Can you work these out from the model? Positions are in its coordinate system, mm. Coordinates: 2 decimals unless noted, no trailing zeros. Loops run counter-clockwise (first coordinate to the right, second up) from the corner with the lowest first, then second, coordinate; pieces in that order, holes last. Notation, with made-up numbers: M -1,17.25 L 57,17.25 A24 cw 57,28.25 Z; hole C 5.5,-11 d9. An arc over 180 degrees is marked long. Answer as a JSON object with one key per item and string values. Group by question number.
Item 1: Suppose I cut it at B-B (z = 21). Write out the boundary of the cut face in (x, y), then the cut area to 3 significant figures.
Item 2: If I drill on line 1 (X direction, y = 1.35, z = 21); line 2 (Y direction, x = 16.5, z = 22.5), over which ranges is the centre line in solid material (lowest first)?
Item 3: I'm going to push a flat-ended pin straight in: pin 1 Ø4.5 at (x, z) = (15, 21) entering from +Y. Where does the tip first touch, or does it pass through?
Item 4: Suppose I cut it at C-C (y = 0.85). Write out the boundary of the cut face in (x, z).
Item 5: We'd pull the mould along Z, two halves only. Please class faces 1 (the flat face through (0, 1, 25.75)), 2 (the cylindrical face through (16.18, 0.89, -22.29)), 3 (the flat face through (-24.75, 1, 0)): +Z half, -Z half, draft (parallel to the pull), parting line (faces both ways), or undercut.
Item 6: Suppose I cut it at A-A (x = 15). Write out the boundary of the cut face in (y, z).
```python
from build123d import *

# Parameters (mm, degrees)
SKETCH1_W           = 49.5
SKETCH1_H           = 51.5
SKETCH1_R           = 1.75
BOSS_EXTRUDE1_DEPTH = 3
CHAMFER1_SIZE       = 1.2
FILLET1_R           = 3


with BuildPart() as part:
    # Sketch1 → Boss-Extrude1 (new body)
    with BuildSketch(Plane(origin=(0, 0, 0), x_dir=(1, 0, 0), z_dir=(0, 1, 0))):
        Rectangle(SKETCH1_W, SKETCH1_H)
        with Locations(Location((-15, 21, 0), (0, 0, 270))):
            Circle(SKETCH1_R, mode=Mode.SUBTRACT)
        with Locations(Location((15, 21, 0), (0, 0, 270))):
            Circle(SKETCH1_R, mode=Mode.SUBTRACT)
        with Locations(Location((-15, -21, 0), (0, 0, 270))):
            Circle(SKETCH1_R, mode=Mode.SUBTRACT)
        with Locations(Location((15, -21, 0), (0, 0, 270))):
            Circle(SKETCH1_R, mode=Mode.SUBTRACT)
    extrude(amount=BOSS_EXTRUDE1_DEPTH)

    # Chamfer1
    chamfer1_edges = [part.edges().sort_by_distance(p)[0] for p in [
        (-15, 3, -22.75),
        (15, 3, -22.75),
        (-15, 3, 19.25),
        (15, 3, 19.25),
    ]]
    chamfer(chamfer1_edges, length=CHAMFER1_SIZE)

    # Fillet1
    fillet1_edges = [part.edges().sort_by_distance(p)[0] for p in [
        (24.75, 1.5, 25.75),
        (-24.75, 1.5, 25.75),
        (-24.75, 1.5, -25.75),
        (24.75, 1.5, -25.75),
    ]]
    fillet(fillet1_edges, radius=FILLET1_R)


solid = part.part
```
From the geometry:
{
 "1": {"outline": "M -24.75,0 L -16.75,0 L -16.75,1.8 L -17.95,3 L -24.75,3 Z; M -13.25,0 L 13.25,0 L 13.25,1.8 L 12.05,3 L -12.05,3 L -13.25,1.8 Z; M 16.75,0 L 24.75,0 L 24.75,3 L 17.95,3 L 16.75,1.8 Z", "area": "125 mm2"},
 "2": {"line 1": "-24.75 to -16.75, -13.25 to 13.25, 16.75 to 24.75", "line 2": "0 to 2.17"},
 "3": {"pin 1": "y = 2.3"},
 "4": {"outline": "M -24.75,-22.75 A3 ccw -21.75,-25.75 L 21.75,-25.75 A3 ccw 24.75,-22.75 L 24.75,22.75 A3 ccw 21.75,25.75 L -21.75,25.75 A3 ccw -24.75,22.75 Z; hole C -15,-21 d3.5; hole C -15,21 d3.5; hole C 15,-21 d3.5; hole C 15,21 d3.5"},
 "5": {"face 1": "+Z half", "face 2": "undercut", "face 3": "draft"},
 "6": {"outline": "M 0,-25.75 L 3,-25.75 L 3,-23.95 L 1.8,-22.75 L 0,-22.75 Z; M 0,-19.25 L 1.8,-19.25 L 3,-18.05 L 3,18.05 L 1.8,19.25 L 0,19.25 Z; M 0,22.75 L 1.8,22.75 L 3,23.95 L 3,25.75 L 0,25.75 Z"}
}
